Part print with two shaded views. Sizes in mm from the minimum x, y, z corner. Round coordinates to 2 decimals unless told otherwise and drop trailing zeros. Loops run counter-clockwise (first coordinate to the right, second up) from the corner with the lowest first, then second, coordinate; pieces in that order, holes last. Notation, with made-up numbers: (-0.5, -25) -> (18.5, -25) arc R12 cw to (18.5, -4) -> close; hole circle Ø11 at (23.25, -17). An arc over 180 degrees is marked (long way). Put each result on its own line as item: value. Start each with the question number.
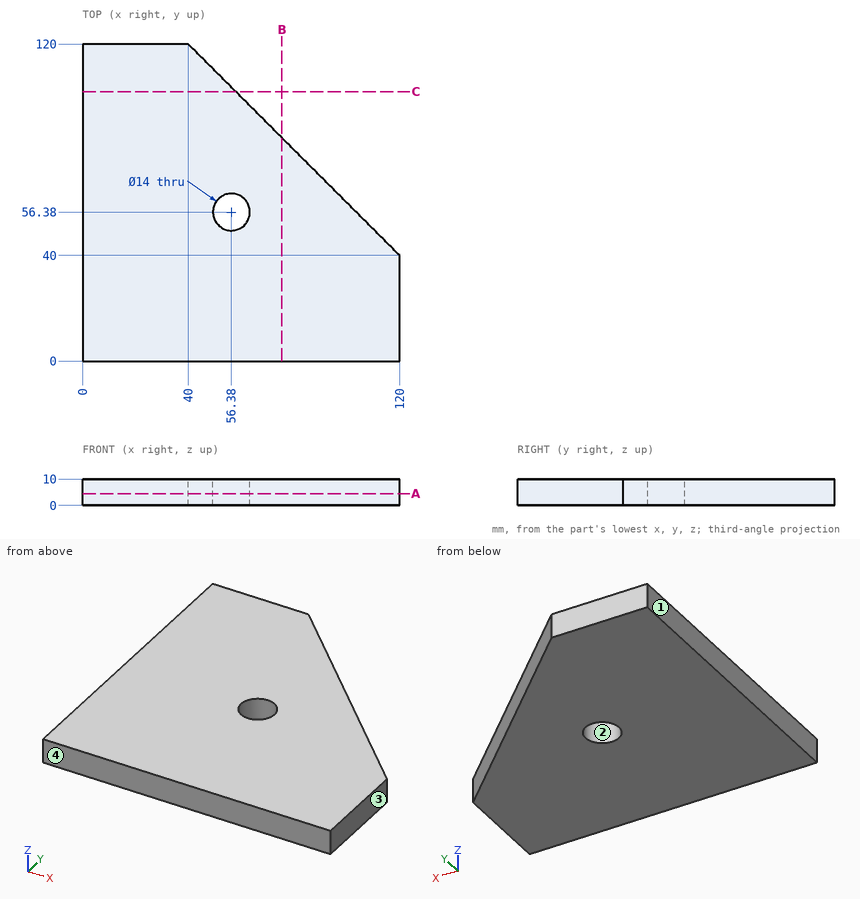
Item 1: Drop flat-ended pins along their axis: pin 1 (6 mm diameter, centred on y = 94, z = 1, fed in from +X); pin 2 (3 mm diameter, centred on x = 55, z = 3, fed in from +Y). Give the stop position or say it passes through.
Item 2: Wall check: line 1 (Y direction, x = 62, z = 7.75) (1 decimal); line 2 (Y direction, x = 54, z = 5.75) (1 decimal); line 3 (X direction, y = 59, z = 2.75). Give the ranges that are in metal, low to high. Write a range as from..to.
Item 3: Cut at C-C on y = 102. Write the cut outline in (x, z).
Item 4: Cut at B-B on x = 75.5. Write the cut outline in (y, z).
Item 5: Cut at A-A on z = 4.5. Write the cut outline in (x, y), then the cut area to 3 significant figures.
Item 6: Pull direction X, two halves, no side cores. Call the marked faces 1, 2, 3 and 4: +X half, -X half, draft (parallel to the pull), parting line (faces both ways), or undercut.
Ans:
1. pin 1: stops at x = 69
1. pin 2: stops at y = 106.5
2. line 1: y = 0..52.2, 60.6..98
2. line 2: y = 0..49.8, 63..106
2. line 3: x = 0..49.89, 62.87..101
3. outline: (0, 0) -> (58, 0) -> (58, 10) -> (0, 10) -> close
4. outline: (0, 0) -> (84.5, 0) -> (84.5, 10) -> (0, 10) -> close
5. outline: (0, 0) -> (120, 0) -> (120, 40) -> (40, 120) -> (0, 120) -> close; hole circle Ø14 at (56.38, 56.38)
5. area: 11,000 mm2
6. face 1: -X half
6. face 2: undercut
6. face 3: +X half
6. face 4: draft
